Geometry: final body of the model. Coordinates: model frame, mm. Face numbers are marked on the shaded views. Give positions to 0.01 mm unless a question says otherwise; leave off trailing zeros. Order: outer loops, then holes, each group sorted by start corner. A loop starts at its lowest first (then second) coordinate and runs counter-clockwise, first axis right, second up. Notation, with made-up numbers: (76, 84) - (102, 84) arc R12 cw to (102, 91) - close; hole circle Ø10 at (49.5, -33.5). An arc over 180 degrees is marked (long way). Use one line per item in the form item = value.
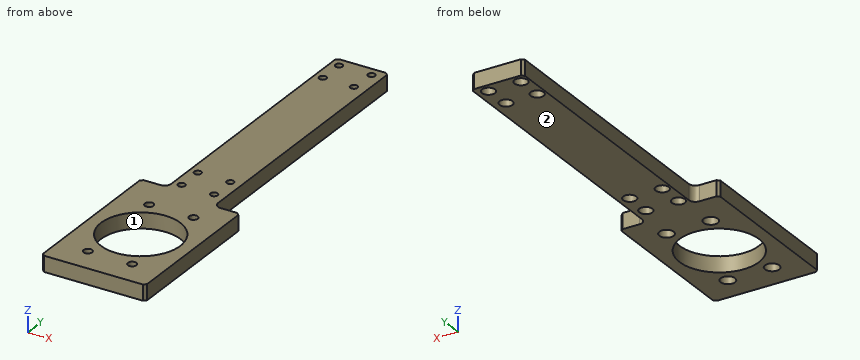
from build123d import *

# Parameters (mm, degrees)
SKETCH_1_W                   = 80
SKETCH_1_H                   = 333.5
EXTRUDE_1_DEPTH              = 12
CHAMFER_1_SIZE               = 2
HOLE_WIZARD_M5_1_D           = 5.5
HOLE_WIZARD_M5_1_CBORE_D     = 10
HOLE_WIZARD_M5_1_CBORE_DEPTH = 5.7
SKETCH_10_W                  = 20
SKETCH_10_H                  = 210
SKETCH_10_H_2                = 216.5
CUT_EXTRUDE_1_DEPTH          = 172.899861838
CHAMFER_2_SIZE               = 2
FILLET_1_R                   = 5
HOLE_WIZARD_M6_1_D           = 6.6
HOLE_WIZARD_M6_1_CBORE_D     = 11
HOLE_WIZARD_M6_1_CBORE_DEPTH = 6.8
SKETCH_14_R                  = 30.5
CUT_EXTRUDE_2_DEPTH          = 172.899861838


with BuildPart() as part:
    # 草图1 → 凸台-拉伸1 (new body)
    with BuildSketch(Plane.XY):
        Rectangle(SKETCH_1_W, SKETCH_1_H)
    extrude(amount=EXTRUDE_1_DEPTH)

    # 倒角1
    chamfer_1_edges = [part.edges().sort_by_distance(p)[0] for p in [
        (-40, -166.75, 6),
        (40, -166.75, 6),
        (40, 166.75, 6),
        (-40, 166.75, 6),
    ]]
    chamfer(chamfer_1_edges, length=CHAMFER_1_SIZE)

    # M5 六角圆柱头螺钉的柱形沉头孔1 (through all)
    with Locations(Plane(origin=(0, 0, 0), x_dir=(-1, 0, 0), z_dir=(0, 0, -1))):
        with Locations((13.5, -35.75), (13.5, 139.25), (-11.5, 159.25), (-10.418856804, 139.25), (13.5, 159.25), (-11.5, -15.75), (13.5, -15.75), (-11.5, -35.75)):
            CounterBoreHole(HOLE_WIZARD_M5_1_D / 2, HOLE_WIZARD_M5_1_CBORE_D / 2, HOLE_WIZARD_M5_1_CBORE_DEPTH)

    # 草图10 → 切除-拉伸1 (cut, through all)
    with BuildSketch(Plane.XY.offset(12)):
        with Locations((-30, 61.75)):
            Rectangle(SKETCH_10_W, SKETCH_10_H)
        with Locations((30, 58.5)):
            Rectangle(SKETCH_10_W, SKETCH_10_H_2)
    extrude(amount=-CUT_EXTRUDE_1_DEPTH, mode=Mode.SUBTRACT)

    # 倒角2
    chamfer_2_edges = [part.edges().sort_by_distance(p)[0] for p in [
        (-40, -43.25, 6),
        (-20, 166.75, 6),
        (40, -49.75, 6),
        (20, 166.75, 6),
    ]]
    chamfer(chamfer_2_edges, length=CHAMFER_2_SIZE)

    # 圆角1
    fillet_1_edges = [part.edges().sort_by_distance(p)[0] for p in [
        (-20, -43.25, 6),
        (20, -49.75, 6),
    ]]
    fillet(fillet_1_edges, radius=FILLET_1_R)

    # M6 六角圆柱头螺钉的柱形沉头孔1 (through all)
    with Locations(Plane(origin=(0, 0, 0), x_dir=(-1, 0, 0), z_dir=(0, 0, -1))):
        with Locations((-17, -70.25), (-17, -146.25), (17, -146.25), (17, -70.25)):
            CounterBoreHole(HOLE_WIZARD_M6_1_D / 2, HOLE_WIZARD_M6_1_CBORE_D / 2, HOLE_WIZARD_M6_1_CBORE_DEPTH)

    # 草图14 → 切除-拉伸2 (cut, through all)
    with BuildSketch(Plane(origin=(0, 0, 0), x_dir=(-1, 0, 0), z_dir=(0, 0, -1))):
        with Locations((0, -108.25)):
            Circle(SKETCH_14_R)
    extrude(amount=-CUT_EXTRUDE_2_DEPTH, mode=Mode.SUBTRACT)


solid = part.part
(1) Contact query for flat-ended pins moving along their axis: pin 1 Ø5 at (x, z) = (25.5, 10.5) entering from +Y; pin 2 Ø3 at (x, y) = (-11.5, -15.5) entering from -Z; pin 3 Ø5 at (y, z) = (-32.5, 5) entering from +X. Output: stop coordinate, or through.
Computed values:
pin_1 = -49.33
pin_2 = 5.7
pin_3 = 20
(2) Pull-direction query (X, two-part tool) for the marked faces 1 and 2; classes: released by +X, released by -X, zero draft, split by the parting line, or undercut.
Computed values:
face_1 = undercut
face_2 = zero draft
(3) Cut plane C-C on x = 0. Output: boundary loops of the cut face in (y, z).
Computed values:
outline = (-166.75, 0) - (-138.75, 0) - (-138.75, 12) - (-166.75, 12) - close; (-77.75, 0) - (166.75, 0) - (166.75, 12) - (-77.75, 12) - close
(4) Cut plane B-B on z = 3.5. Give the number of separate pieces and of enclosed holes in the cut face, plus the area to 3 significant figures.
Computed values:
separate_pieces = 1
enclosed_holes = 13
area = 14,200 mm²
(5) Ray query, line 1 along X through (y, z) = (-146.25, 8.55); line 2 along X through (y, z) = (139.25, 10.5); line 3 along Y through (x, z) = (19.5, 2). Return the intervals inside material, ascending.
Computed values:
line_1 = -40 to -20.3, -13.7 to 13.7, 20.3 to 40
line_2 = -20 to -16.25, -10.75 to 7.67, 13.17 to 20
line_3 = -166.75 to -151.15, -141.35 to -131.7, -84.8 to -75.15, -65.35 to 165.25
(6) Cut plane D-D on y = -146.25. Output: boundary loops of the cut face in (x, z), plus the area to 3 significant figures.
Computed values:
outline = (-40, 0) - (-22.5, 0) - (-22.5, 6.8) - (-20.3, 6.8) - (-20.3, 12) - (-40, 12) - close; (-13.7, 6.8) - (-11.5, 6.8) - (-11.5, 0) - (11.5, 0) - (11.5, 6.8) - (13.7, 6.8) - (13.7, 12) - (-13.7, 12) - close; (20.3, 6.8) - (22.5, 6.8) - (22.5, 0) - (40, 0) - (40, 12) - (20.3, 12) - close
area = 742 mm²
(7) Cut plane A-A on y = -15.75. Output: boundary loops of the cut face in (x, z), plus the area to 3 significant figures.
Computed values:
outline = (-20, 0) - (-18.5, 0) - (-18.5, 5.7) - (-16.25, 5.7) - (-16.25, 12) - (-20, 12) - close; (-10.75, 5.7) - (-8.5, 5.7) - (-8.5, 0) - (6.5, 0) - (6.5, 5.7) - (8.75, 5.7) - (8.75, 12) - (-10.75, 12) - close; (14.25, 5.7) - (16.5, 5.7) - (16.5, 0) - (20, 0) - (20, 12) - (14.25, 12) - close
area = 297 mm²
